```python
from build123d import *

# Parameters (mm, degrees)
BASE_PLATE_SKETCH_W            = 60
BASE_PLATE_SKETCH_H            = 100
BASE_PLATE_100X60X12_DEPTH     = 12
PEDESTAL_SKETCH_W              = 60
PEDESTAL_SKETCH_H              = 60
TAPERED_PEDESTAL_DEPTH         = 28
TAPERED_PEDESTAL_TAPER         = 10
FOOT_CHANNEL_SKETCH_W          = 30
FOOT_CHANNEL_SKETCH_H          = 12
FOOT_CHANNEL_CUT_DEPTH         = 200
UPPER_BLOCK_SKETCH_W           = 50.13
UPPER_BLOCK_SKETCH_H           = 80
UPPER_BLOCK_80X50_DEPTH        = 16
UPPER_BLOCK_80X50_TAPER        = 10
TOP_SLOT_SKETCH_W              = 24
TOP_SLOT_SKETCH_H              = 8.960181453
TOP_SLOT_CUT_DEPTH             = 16
PEDESTAL_RELIEF_SKETCH_W       = 30
PEDESTAL_RELIEF_SKETCH_H       = 60
PEDESTAL_RELIEF_CUT_DEPTH      = 50
PEDESTAL_RELIEF_CUT_DRAFT      = -10
WINDOW_SKETCH_W                = 24
WINDOW_SKETCH_H                = 20
SQUARE_WINDOW_20X20_DEPTH      = 5
SIDE_POCKET_SKETCH_W           = 24
SIDE_POCKET_SKETCH_H           = 8.960181453
SIDE_POCKET_SKETCH_H_2         = 11.039818547
SIDE_POCKET_CUT_DEPTH          = 20
RIB_BOSS_SKETCH_W              = 44.487536618
RIB_BOSS_SKETCH_H              = 74.357536618
RIB_BOSS_DEPTH                 = 20
RIB_BOSS_TAPER                 = 10
TRIM_CUT_DEPTH                 = 100
UPRIGHTS_SKETCH_W              = 44.487536618
UPRIGHTS_SKETCH_H              = 15
UPRIGHTS_15X15_DEPTH           = 20
UPRIGHTS_15X15_DRAFT           = 1
UPRIGHTS_15X15_PROFILE_2_DEPTH = 20
UPRIGHTS_15X15_PROFILE_2_DRAFT = 1
CRADLE_CUT_A_DEPTH             = 200
CRADLE_CUT_B_DEPTH             = 200
CROSS_BORE_CUT_DEPTH           = 100


with BuildPart() as part:
    # Base Plate Sketch → Base Plate 100x60x12 (new body)
    with BuildSketch(Plane(origin=(0, 0, 0), x_dir=(1, 0, 0), z_dir=(0, 1, 0))):
        Rectangle(BASE_PLATE_SKETCH_W, BASE_PLATE_SKETCH_H)
    extrude(amount=BASE_PLATE_100X60X12_DEPTH)

    # Pedestal Sketch → Tapered Pedestal (add)
    with BuildSketch(Plane(origin=(0, 12, 0), x_dir=(1, 0, 0), z_dir=(0, 1, 0))):
        Rectangle(PEDESTAL_SKETCH_W, PEDESTAL_SKETCH_H)
    extrude(amount=TAPERED_PEDESTAL_DEPTH, taper=TAPERED_PEDESTAL_TAPER)

    # Foot Channel Sketch → Foot Channel Cut (cut)
    with BuildSketch(Plane.XY.offset(50)):
        with BuildLine():
            ThreePointArc((15, 12), (0, 27), (-15, 12))
            Line((-15, 12), (15, 12))
        make_face()
        with Locations((0, 6)):
            Rectangle(FOOT_CHANNEL_SKETCH_W, FOOT_CHANNEL_SKETCH_H)
    extrude(amount=-FOOT_CHANNEL_CUT_DEPTH, mode=Mode.SUBTRACT)

    # Upper Block Sketch → Upper Block 80x50 (add)
    with BuildSketch(Plane(origin=(0, 40, 0), x_dir=(1, 0, 0), z_dir=(0, 1, 0))):
        Rectangle(UPPER_BLOCK_SKETCH_W, UPPER_BLOCK_SKETCH_H)
    extrude(amount=UPPER_BLOCK_80X50_DEPTH, taper=UPPER_BLOCK_80X50_TAPER)

    # Top Slot Sketch → Top Slot Cut (cut)
    with BuildSketch(Plane(origin=(31.149600637, 5.492515031, 0), x_dir=(0, 0, -1), z_dir=(0.9848077530122081, 0.17364817766693072, 0))):
        with Locations((0, 39.519909274)):
            Rectangle(TOP_SLOT_SKETCH_W, TOP_SLOT_SKETCH_H)
        Polygon((-12, 35.039818547), (-12, 24), (0, 24), (12, 24), (12, 35.039818547), align=None)
    extrude(amount=-TOP_SLOT_CUT_DEPTH, mode=Mode.SUBTRACT)


with BuildPart() as pedestal_relief_cut_tool:
    # Pedestal Relief Sketch → Pedestal Relief Cut (with draft: the straight prism first)
    with BuildSketch(Plane.XZ):
        Rectangle(PEDESTAL_RELIEF_SKETCH_W, PEDESTAL_RELIEF_SKETCH_H)
    extrude(amount=-PEDESTAL_RELIEF_CUT_DEPTH)
    # Pedestal Relief Cut: the draft: its side faces are tilted about the plane it starts from
    pedestal_relief_cut_sides = [pedestal_relief_cut_tool.faces().sort_by_distance(p)[0] for p in [
        (-15, 25, 0),
        (0, 25, -30),
        (15, 25, 0),
        (0, 25, 30),
    ]]
    draft(pedestal_relief_cut_sides, Plane.XZ, PEDESTAL_RELIEF_CUT_DRAFT)


with BuildPart() as part_1:
    add(part.part)

    # Pedestal Relief Cut: cut by pedestal_relief_cut_tool
    add(pedestal_relief_cut_tool.part, mode=Mode.SUBTRACT)

    # Window Sketch → Square Window 20x20 (cut)
    with BuildSketch(Plane(origin=(15.392676588, 2.714144188, 0), x_dir=(0, 0, -1), z_dir=(0.9848077530122081, 0.1736481776669307, 0))):
        with Locations((0, 34)):
            Rectangle(WINDOW_SKETCH_W, WINDOW_SKETCH_H)
    extrude(amount=-SQUARE_WINDOW_20X20_DEPTH, mode=Mode.SUBTRACT)

    # Side Pocket Sketch → Side Pocket Cut (cut)
    with BuildSketch(Plane(origin=(-31.149600637, 5.492515031, 0), x_dir=(0, 0, 1), z_dir=(-0.9848077530122081, 0.17364817766693072, 0))):
        with Locations((0, 39.519909274)):
            Rectangle(SIDE_POCKET_SKETCH_W, SIDE_POCKET_SKETCH_H)
        with Locations((0, 29.519909274)):
            Rectangle(SIDE_POCKET_SKETCH_W, SIDE_POCKET_SKETCH_H_2)
    extrude(amount=-SIDE_POCKET_CUT_DEPTH, mode=Mode.SUBTRACT)

    # Rib Boss Sketch → Rib Boss (add)
    with BuildSketch(Plane(origin=(0, 56, 0), x_dir=(1, 0, 0), z_dir=(0, 1, 0))):
        Rectangle(RIB_BOSS_SKETCH_W, RIB_BOSS_SKETCH_H)
    extrude(amount=RIB_BOSS_DEPTH, taper=RIB_BOSS_TAPER)

    # Trim Sketch → Trim Cut (cut)
    with BuildSketch(Plane.XY.offset(50)):
        Polygon((0, 56), (24.962521637, 56), (24.962521637, 76), (-29.161824343, 76), (-29.161824343, 56), align=None)
    extrude(amount=-TRIM_CUT_DEPTH, mode=Mode.SUBTRACT)


with BuildPart() as uprights_15x15_tool:
    # Uprights Sketch → Uprights 15x15 (with draft: the straight prism first)
    with BuildSketch(Plane(origin=(0, 56, 0), x_dir=(1, 0, 0), z_dir=(0, 1, 0))):
        with Locations((0, 29.678768309)):
            Rectangle(UPRIGHTS_SKETCH_W, UPRIGHTS_SKETCH_H)
    extrude(amount=UPRIGHTS_15X15_DEPTH)
    # Uprights 15x15: the draft: its side faces are tilted about the plane it starts from
    uprights_15x15_sides = [uprights_15x15_tool.faces().sort_by_distance(p)[0] for p in [
        (-22.243768309, 66, -29.678768309),
        (0, 66, -22.178768309),
        (22.243768309, 66, -29.678768309),
        (0, 66, -37.178768309),
    ]]
    draft(uprights_15x15_sides, Plane(origin=(0, 56, 0), x_dir=(1, 0, 0), z_dir=(0, 1, 0)), UPRIGHTS_15X15_DRAFT)


with BuildPart() as part_2:
    add(part_1.part)

    # Uprights 15x15: add uprights_15x15_tool
    add(uprights_15x15_tool.part)


with BuildPart() as uprights_15x15_profile_2_tool:
    # Uprights Sketch → Uprights 15x15 profile 2 (with draft: the straight prism first)
    with BuildSketch(Plane(origin=(0, 56, 0), x_dir=(1, 0, 0), z_dir=(0, 1, 0))):
        with Locations((0, -29.678768309)):
            Rectangle(UPRIGHTS_SKETCH_W, UPRIGHTS_SKETCH_H)
    extrude(amount=UPRIGHTS_15X15_PROFILE_2_DEPTH)
    # Uprights 15x15 profile 2: the draft: its side faces are tilted about the plane it starts from
    uprights_15x15_profile_2_sides = [uprights_15x15_profile_2_tool.faces().sort_by_distance(p)[0] for p in [
        (0, 66, 37.178768309),
        (22.243768309, 66, 29.678768309),
        (0, 66, 22.178768309),
        (-22.243768309, 66, 29.678768309),
    ]]
    draft(uprights_15x15_profile_2_sides, Plane(origin=(0, 56, 0), x_dir=(1, 0, 0), z_dir=(0, 1, 0)), UPRIGHTS_15X15_PROFILE_2_DRAFT)


with BuildPart() as part_3:
    add(part_2.part)

    # Uprights 15x15 profile 2: add uprights_15x15_profile_2_tool
    add(uprights_15x15_profile_2_tool.part)

    # Cradle Cut A Sketch → Cradle Cut A (cut)
    with BuildSketch(Plane.XY.offset(50)):
        Polygon((20, 76), (22.243768309, 56), (21.89466701, 76), align=None)
        Polygon((-22.243768309, 56), (-20, 76), (-21.89466701, 76), align=None)
    extrude(amount=-CRADLE_CUT_A_DEPTH, mode=Mode.SUBTRACT)

    # Cradle Cut B Sketch → Cradle Cut B (cut)
    with BuildSketch(Plane(origin=(30, 0, 0), x_dir=(0, 0, -1), z_dir=(1, 0, 0))):
        Polygon((-40, 40), (-33.208201883, 76), (-36.82966701, 76), align=None)
        Polygon((40, 40), (33.445403325, 76), (36.82966701, 76), align=None)
    extrude(amount=-CRADLE_CUT_B_DEPTH, mode=Mode.SUBTRACT)

    # Cross Bore Sketch → Cross Bore Cut (cut)
    with BuildSketch(Plane.XY.offset(50)):
        with BuildLine():
            Line((-10, 76), (10, 76))
            ThreePointArc((10, 76), (0, 66), (-10, 76))
        make_face()
    extrude(amount=-CROSS_BORE_CUT_DEPTH, mode=Mode.SUBTRACT)


solid = part_3.part
```
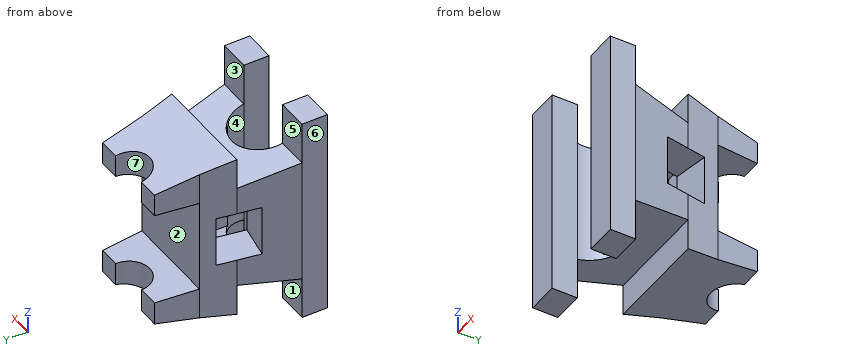
Can you work these out from the model? Positions are in its coordinate system, mm. Face numbers are marked on the shaded views. A direction names the side the tool comes from. Coordinates: 2 decimals unless noted, no trailing zeros. Loops run counter-clockwise (first coordinate to the right, second up) from the corner with the lowest first, then second, coordinate; pieces in that order, holes last.
1) Imagine slicing it at A-A on z = 31.5. List the corners of the cut face in (x, y) for me (3 decimals), plus the area to 3 significant figures.
2) Thinking about a two-plate mould opening in Y: for the marked faces 4, 5, 6 and 7, which applies, pulls with the +Y half, pulls with the -Y half, needs draft (parallel to the pull), parting line crosses it, or undercut?
3) Which directions (+Z, -Z, +X, -X, +Y, -Y) give clear straight access to the entire face, cutting with the end or side of a thin tool? Please do the marked faces 1, 2 and 3.
4) Imagine slicing it at B-B on y = 69. List the corners of the cut face in (x, z) for me.
5) I need wall thicknesses on probe 1 along X at (y, z) = (10.5, 40); probe 2 along Y at (x, z) = (-15.5, -1.5); probe 3 along X at (y, z) = (23, -13). Which ranges of each line are inside material? Lowest first, please.
6) Imagine slicing it at C-C on z = 1. State how many separate pieces and enclosed holes the cut face has, plus the area to 3 significant figures.
7) For pin 1 (1 mm diameter, centred on y = 46.5, z = -38.5, fed in from +X); pin 2 (22 mm diameter, centred on x = 15.5, y = 40.5, fed in from +Z); pin 3 (22 mm diameter, centred on x = -21, y = 32.5, fed in from -Z); pin 4 (12 mm diameter, centred on x = -22.5, z = -35.5, fed in from +Y), each with a flat end and sliding along its axis, tell me the tip position at first contact or that it passes through.
Completed:
1. outline: (-30, 0) - (-15, 0) - (-15, 12) - (-30, 12) - close; (-25.065, 40) - (25.065, 40) - (22.244, 56) - (20, 76) - (10, 76) arc R10 cw to (-10, 76) - (-20, 76) - (-22.244, 56) - close; (15, 0) - (30, 0) - (30, 12) - (15, 12) - close
1. area: 1,800 mm2
2. face 4: pulls with the -Y half
2. face 5: undercut
2. face 6: needs draft
2. face 7: pulls with the +Y half
3. face 1: -Z, +X, -X
3. face 2: +X, -X, +Y
3. face 3: +Z, +X, -X
4. outline: (-20.79, -34.72) - (-7.14, -34.72) - (-7.14, -22.41) - (-20.79, -22.41) - close; (-20.79, 22.41) - (-7.14, 22.41) - (-7.14, 34.53) - (-20.79, 34.53) - close; (7.14, -34.72) - (20.79, -34.72) - (20.79, -22.41) - (7.14, -22.41) - close; (7.14, 22.41) - (20.79, 22.41) - (20.79, 34.53) - (7.14, 34.53) - close
5. probe 1: x = -30 to -15, 15 to 30
5. probe 2: y = 0 to 27.1, 47.41 to 56
5. probe 3: x = -28.06 to -10.94, 10.94 to 28.06
6. separate pieces: 3
6. enclosed holes: 0
6. area: 1,220 mm2
7. pin 1: stops at x = 24.01
7. pin 2: stops at z = 40
7. pin 3: stops at z = -40
7. pin 4: stops at y = 76
